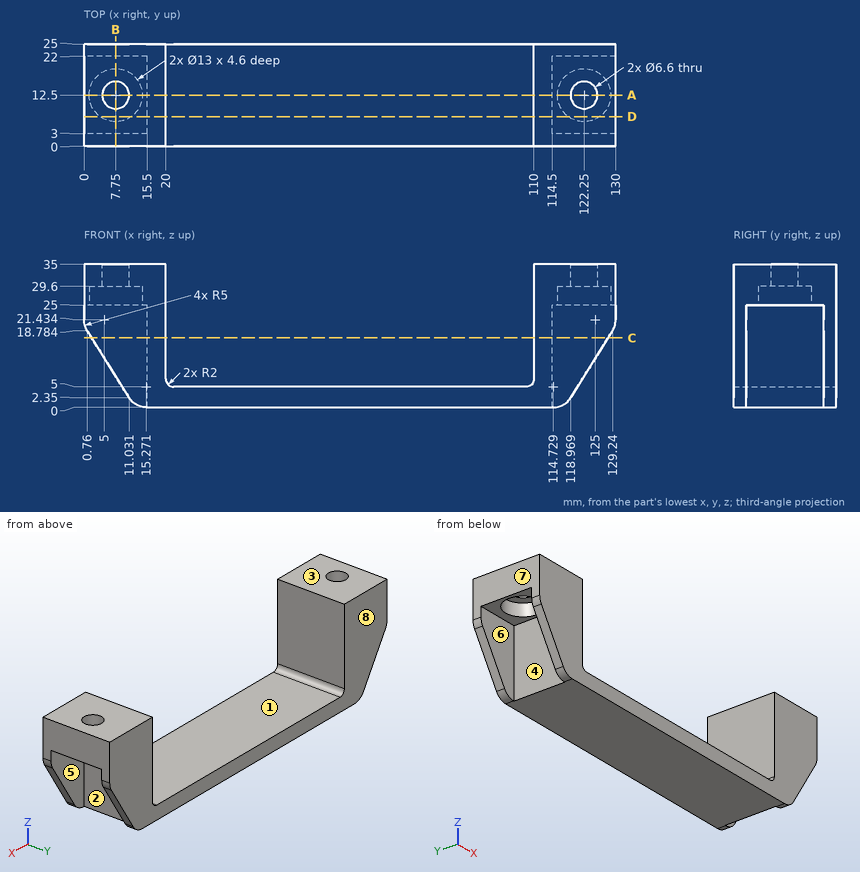
Verification items for this drawing (mm, ordinates from the low corner). A direction names the side the tool comes from. Coordinates: 2 decimals unless noted, no trailing zeros. Loops run counter-clockwise (first coordinate to the right, second up) from the corner with the lowest first, then second, coordinate; pieces in that order, holes last. Notation, with made-up numbers: (6.25, 27.25) - (27.25, 27.25) arc R9 ccw to (27.25, 44.25) - close; hole circle Ø9 at (55.5, 47). An arc over 180 degrees is marked (long way). Answer as a JSON object with one key per item and string values.
(1) Cross-section at C-C, the plane z = 17. Record the boundary of the cut face in (x, y) (1 decimal).
Response:
{"outline": "(1.9, 0) - (20, 0) - (20, 25) - (1.9, 25) - (1.9, 22) - (15.5, 22) - (15.5, 3) - (1.9, 3) - close; (110, 0) - (128.1, 0) - (128.1, 3) - (114.5, 3) - (114.5, 22) - (128.1, 22) - (128.1, 25) - (110, 25) - close"}
(2) Go/stop test with flat-tipped pins: pin 1 Ø5 at (y, z) = (15, 24) entering from -X; pin 2 Ø15 at (x, y) = (122.25, 12.5) entering from -Z; pin 3 Ø6 at (x, y) = (84.5, 20.5) entering from +Z; pin 4 Ø5.5 at (y, z) = (12, 6.5) entering from +X. Record where each tip stops, or that it passes through.
Response:
{"pin 1": "stops at x = 0", "pin 2": "stops at z = 25", "pin 3": "stops at z = 5", "pin 4": "stops at x = 114.5"}
(3) Cross-section at D-D, the plane y = 7.25. Record the boundary of the cut face in (x, z), then the cut area to 3 significant figures.
Response:
{"outline": "(0, 25) - (3.92, 25) - (3.92, 29.6) - (11.58, 29.6) - (11.58, 25) - (15.5, 25) - (15.5, 0) - (114.5, 0) - (114.5, 25) - (118.42, 25) - (118.42, 29.6) - (126.08, 29.6) - (126.08, 25) - (130, 25) - (130, 35) - (110, 35) - (110, 7) arc R2 cw to (108, 5) - (22, 5) arc R2 cw to (20, 7) - (20, 35) - (0, 35) - close", "area": "1,010 mm²"}
(4) Cross-section at B-B, the plane x = 7.75. Record the boundary of the cut face in (y, z), then the cut area to 3 significant figures.
Response:
{"outline": "(0, 7.6) - (3, 7.6) - (3, 25) - (6, 25) - (6, 29.6) - (9.2, 29.6) - (9.2, 35) - (0, 35) - close; (15.8, 29.6) - (19, 29.6) - (19, 25) - (22, 25) - (22, 7.6) - (25, 7.6) - (25, 35) - (15.8, 35) - close", "area": "259 mm²"}
(5) Access from +Z, -Z, +X, -X, +Y, -Y to the whole of each face (thin tool, end or side, straight path). Record for the marked faces 1, 2, 3 and 4.
Response:
{"face 1": "+Z, +Y, -Y", "face 2": "-Z, +X", "face 3": "+Z, +X, -X, +Y, -Y", "face 4": "-Z, -X"}
(6) Scan lines: line 1 along X through (y, z) = (19.75, 22.5); line 2 along Y through (x, z) = (122.25, 32.65); line 3 along Y through (x, z) = (13, 5.5). Record each from-to range of solid material in increasing order.
Response:
{"line 1": "x = 15.5 to 20, 110 to 114.5", "line 2": "y = 0 to 9.2, 15.8 to 25", "line 3": "y = 0 to 3, 22 to 25"}
(7) Cross-section at A-A, the plane y = 12.5. Count the separate pieces of the cut face and the enclosed holes in it, then the cut area to 3 significant figures.
Response:
{"separate pieces": "3", "enclosed holes": "0", "area": "886 mm²"}
(8) Mould release check, pull along Y, two halves, no side actions. Record for the marked faces 5, 6, 7 and 8: pulls with the +Y half, pulls with the -Y half, needs draft (parallel to the pull), parting line crosses it, or undercut.
Response:
{"face 5": "undercut", "face 6": "undercut", "face 7": "needs draft", "face 8": "pulls with the +Y half"}
